Input: dimensioned drawing with shaded views. Units: mm. Origin: part minimum x, y, z. Round coordinates to 2 decimals unless told otherwise and drop trailing zeros. Write each loop counter-clockwise with the first axis right and the second up, starting at its lowest first coordinate (ties: lowest second). Pieces come first, ordered by that corner, then holes. Notation, with made-up numbers: (1.5, 9.25) -> (5.5, 9.25) arc R23 ccw to (5.5, 23.25) -> close; hole circle Ø11 at (36, 0.5). An arc over 180 degrees is marked (long way). Use one line per item in the form item = value. Start each with the question number.
1. Cut plane A-A, the plane z = 2.45. Return the cut outline in (x, y).
2. Cut plane B-B, the plane y = 34. Return the cut outline in (x, z), plus the area to 3 significant figures.
3. Pin query (flat end, axial travel): pin 1 Ø2 at (x, y) = (9.5, 22) entering from -Z; pin 2 Ø1.5 at (y, z) = (40, 1) entering from +X; pin 3 Ø0.9 at (x, z) = (38.5, 1.5) entering from +Y. Return the tip coordinate at first contact, or that it passes through.
4. Line query: L1, parallel to X at y = 42, z = 2.6. Output: solid intervals per line, ascending.
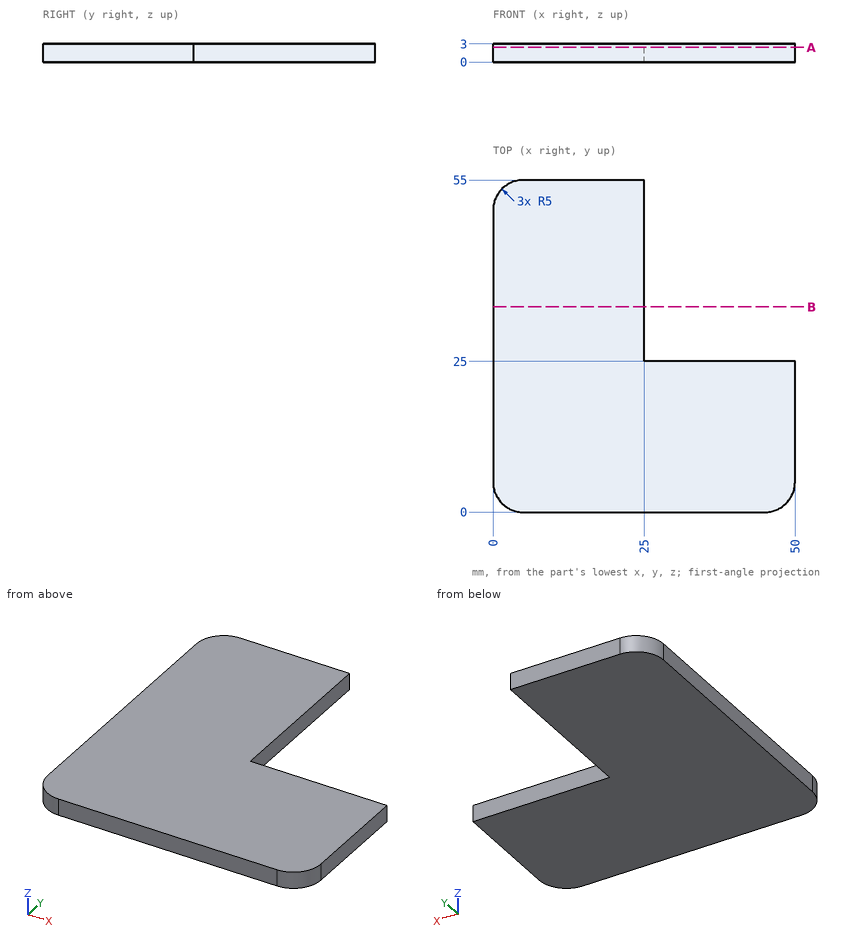
Outcome:
q1.outline = (0, 5) arc R5 ccw to (5, 0) -> (45, 0) arc R5 ccw to (50, 5) -> (50, 25) -> (25, 25) -> (25, 55) -> (5, 55) arc R5 ccw to (0, 50) -> close
q2.outline = (0, 0) -> (25, 0) -> (25, 3) -> (0, 3) -> close
q2.area = 75.0 mm^2
q3.pin_1 = 0
q3.pin_2 = 25
q3.pin_3 = 25
q4.L1 = 0 to 25
